from build123d import *

# Parameters (mm, degrees)
SKETCH2_R          = 3.5
CUT_EXTRUDE1_DEPTH = 47.368092477
CUT_EXTRUDE2_DEPTH = 47.368092477


with BuildPart() as part:
    # Sketch1 → Revolve1 (revolve)
    with BuildSketch(Plane.XY, mode=Mode.PRIVATE) as revolve1_sk:
        Polygon((12, 36), (12, 0), (25, 0), (25, 6), (16, 6), (16, 36), align=None)
    revolve(revolve1_sk.sketch.rotate(Axis((0, 0, 0), (0, 1, 0)), 90), axis=Axis((0, 0, 0), (0, 1, 0)))

    # Sketch2 → Cut-Extrude1 (cut, through all)
    with BuildSketch(Plane(origin=(0, 6, 0), x_dir=(1, 0, 0), z_dir=(0, 1, 0))):
        with Locations(Location((-20.5, 0, 0), (0, 0, 270))):
            Circle(SKETCH2_R)
        with Locations(Location((0, 20.5, 0), (0, 0, 270))):
            Circle(SKETCH2_R)
        with Locations(Location((20.5, 0, 0), (0, 0, 270))):
            Circle(SKETCH2_R)
        with Locations(Location((0, -20.5, 0), (0, 0, 270))):
            Circle(SKETCH2_R)
    extrude(amount=-CUT_EXTRUDE1_DEPTH, mode=Mode.SUBTRACT)

    # Sketch3 → Cut-Extrude2 (cut, through all)
    with BuildSketch(Plane(origin=(0, 6, 0), x_dir=(1, 0, 0), z_dir=(0, 1, 0))):
        with BuildLine():
            Line((-19.209372712, 16), (19.209372712, 16))
            ThreePointArc((19.209372712, 16), (0, 25), (-19.209372712, 16))
        make_face()
        with BuildLine():
            Line((-19.209372712, -16), (19.209372712, -16))
            ThreePointArc((19.209372712, -16), (0, -25), (-19.209372712, -16))
        make_face()
    extrude(amount=-CUT_EXTRUDE2_DEPTH, mode=Mode.SUBTRACT)


solid = part.part
Design review of the part built by this model. Coordinates are the model's own, in mm. A direction names the side the tool comes from. Round coordinates to 2 decimals unless told otherwise and drop trailing zeros. Write each loop counter-clockwise with the first axis right and the second up, starting at its lowest first coordinate (ties: lowest second). Pieces come first, ordered by that corner, then holes. Notation, with made-up numbers: (54, 63) -> (64, 63) arc R24 cw to (64, 101) -> close; hole circle Ø8 at (44.25, 37). An arc over 180 degrees is marked (long way). One line per item, written item: value. Start each with the question number.
Q1. Insertion check: P1, Ø3, axis at y = 28.5, z = 8.5, coming from the +X side; P2, Ø6, axis at y = 27, z = 4, coming from the +X side; P3, Ø5.5, axis at x = -20.5, z = 0, coming from the -Y side; P4, Ø12, axis at x = -11, z = -3, coming from the +Y side. Each pin has a flat end and moves straight along its axis. Give the tip position at first contact, or say it passes through.
Q2. Add section A-A (x = 20.5). Give the boundary of the cut face in (y, z).
Q3. Add section B-B (z = 0). Give the boundary of the cut face in (x, y), then the cut area to 3 significant figures.
Q4. Tool access review of faces 4 (the face through (-18, 6, 4)), 5 (the face through (18, 6, -3)), 6 (the face through (25, 3, 0)): name each direction out of +Z, -Z, +X, -X, +Y, -Y from which nothing blocks a thin tool from reaching the whole face with its end or side.
Q5. To check wall thickness, follow probe 1 along X at (y, z) = (3, 0); probe 2 along X at (y, z) = (3, 3); probe 3 along Y at (x, z) = (16.5, -3). State the ranges of each line that lie inside material, in increasing order.
Q6. The part is to be moulded in two halves that separate along X. For faces 1 (the face through (-12, 36, -2)), 2 (the face through (-3.604, 17.748, -11.446)), 3 (the face through (15.62, 21.21, 3.47)), say which applies: pulls with the +X half, pulls with the -X half, needs draft (parallel to the pull), parting line crosses it, or undercut.
Q7. Add section D-D (y = 10.5). Give the boundary of the cut face in (x, z).
Q8. Add section C-C (z = -8.5). Give the boundary of the cut face in (x, y).
Response:
1. P1: stops at x = 14.39
1. P2: stops at x = 15.97
1. P3: passes through
1. P4: stops at y = 36
2. outline: (0, -14.31) -> (6, -14.31) -> (6, -3.5) -> (0, -3.5) -> close; (0, 3.5) -> (6, 3.5) -> (6, 14.31) -> (0, 14.31) -> close
3. outline: (-25, 0) -> (-24, 0) -> (-24, 6) -> (-25, 6) -> close; (-17, 0) -> (-12, 0) -> (-12, 36) -> (-16, 36) -> (-16, 6) -> (-17, 6) -> close; (12, 0) -> (17, 0) -> (17, 6) -> (16, 6) -> (16, 36) -> (12, 36) -> close; (24, 0) -> (25, 0) -> (25, 6) -> (24, 6) -> close
3. area: 312 mm^2
4. face 4: -X, +Y
4. face 5: +X, +Y
4. face 6: +X, +Y, -Y
5. probe 1: x = -25 to -24, -17 to -12, 12 to 17, 24 to 25
5. probe 2: x = -24.82 to -22.3, -18.7 to -11.62, 11.62 to 18.7, 22.3 to 24.82
5. probe 3: y = 0 to 6
6. face 1: needs draft
6. face 2: undercut
6. face 3: parting line crosses it
7. outline: circle Ø32 at (0, 0); hole circle Ø24 at (0, 0)
8. outline: (-23.51, 0) -> (-8.47, 0) -> (-8.47, 36) -> (-13.56, 36) -> (-13.56, 6) -> (-23.51, 6) -> close; (8.47, 0) -> (23.51, 0) -> (23.51, 6) -> (13.56, 6) -> (13.56, 36) -> (8.47, 36) -> close
